Check sheet for the modelled part. Datum: model origin and axes. Units: mm. A direction names the side the tool comes from. Give positions to 0.01 mm unless a question says otherwise; leave off trailing zeros. Order: outer loops, then holes, each group sorted by start corner. A loop starts at its lowest first (then second) coordinate and runs counter-clockwise, first axis right, second up.
```python
from build123d import *

# Parameters (mm, degrees)
SKETCH2_R           = 5
BOSS_EXTRUDE1_DEPTH = 10.5
SKETCH3_R           = 2.5
CUT_EXTRUDE1_DEPTH  = 3.5
SKETCH4_R           = 1
CUT_EXTRUDE2_DEPTH  = 10.949874371
SKETCH5_W           = 1.25
SKETCH5_H           = 6
CUT_EXTRUDE3_DEPTH  = 16.33786165
SKETCH6_W           = 2.3
SKETCH6_H           = 6
CUT_EXTRUDE4_DEPTH  = 16.33786165
SKETCH7_R           = 2.6
CUT_EXTRUDE5_DEPTH  = 6
SKETCH8_R           = 0.5
CUT_EXTRUDE6_DEPTH  = 15.553779578


with BuildPart() as part:
    # Sketch2 → Boss-Extrude1 (new body)
    with BuildSketch(Plane.XY):
        with Locations(Location((0, 0, 0), (0, 0, 180))):
            Circle(SKETCH2_R)
    extrude(amount=BOSS_EXTRUDE1_DEPTH)

    # Sketch3 → Cut-Extrude1 (cut)
    with BuildSketch(Plane(origin=(0, 0, 0), x_dir=(-1, 0, 0), z_dir=(0, 0, -1))):
        Circle(SKETCH3_R)
    extrude(amount=-CUT_EXTRUDE1_DEPTH, mode=Mode.SUBTRACT)

    # Sketch4 → Cut-Extrude2 (cut, through all)
    with BuildSketch(Plane(origin=(0, 0, 3.5), x_dir=(-1, 0, 0), z_dir=(0, 0, -1))):
        Circle(SKETCH4_R)
    extrude(amount=-CUT_EXTRUDE2_DEPTH, mode=Mode.SUBTRACT)

    # Sketch5 → Cut-Extrude3 (cut, through all)
    with BuildSketch(Plane(origin=(0, 5, 0), x_dir=(1, 0, 0), z_dir=(0, 1, 0))):
        with Locations((-4.375, -7.5)):
            Rectangle(SKETCH5_W, SKETCH5_H)
        with Locations((4.375, -7.5)):
            Rectangle(SKETCH5_W, SKETCH5_H)
    extrude(amount=-CUT_EXTRUDE3_DEPTH, mode=Mode.SUBTRACT)

    # Sketch6 → Cut-Extrude4 (cut, through all)
    with BuildSketch(Plane(origin=(0, 5, 0), x_dir=(1, 0, 0), z_dir=(0, 1, 0))):
        with Locations((0, -7.5)):
            Rectangle(SKETCH6_W, SKETCH6_H)
    extrude(amount=-CUT_EXTRUDE4_DEPTH, mode=Mode.SUBTRACT)

    # Sketch7 → Cut-Extrude5 (cut)
    with BuildSketch(Plane.XY.offset(10.5)):
        Circle(SKETCH7_R)
    extrude(amount=-CUT_EXTRUDE5_DEPTH, mode=Mode.SUBTRACT)

    # Sketch8 → Cut-Extrude6 (cut, through all)
    with BuildSketch(Plane.ZY.offset(3.75)):
        with Locations((8, 1.85)):
            Circle(SKETCH8_R)
        with Locations((8, -1.85)):
            Circle(SKETCH8_R)
    extrude(amount=-CUT_EXTRUDE6_DEPTH, mode=Mode.SUBTRACT)


solid = part.part
```
Q1. Sectioned sample at B-B, the plane z = 9.5. Record the cut outline in (x, y), plus the area to 3 significant figures.
Q2. Material ranges on line 1 (Z direction, x = 2.6, y = -1.85); line 2 (Y direction, x = 0, z = 0.8); line 3 (X direction, y = -3, z = 8.5), recorded low to high.
Q3. Sectioned sample at C-C, the plane y = 0. Record the cut outline in (x, z), plus the area to 3 significant figures.
Q4. Sectioned sample at A-A, the plane x = 0. Record the cut outline in (y, z).
Q5. Tool access check on faces 4 (the flat face through (-3.75, 0, 8)), 5 (the cylindrical face through (-2.6, 0, 7.5)), 6 (the flat face through (1.15, 4, 8)), 7 (the flat face through (4, 0, 4.5)), 8 (the flat face through (-1, -1, 3.5)). Record the directions out of +Z, -Z, +X, -X, +Y, -Y that give a thin tool (end or side, any length) a straight path to the whole face; none if there is none.
Q6. Draft check along Y on faces 1 (the cylindrical face through (-3, -4, 4)), 2 (the flat face through (-3, 0, 10.5)), 3 (the cylindrical face through (2.721, 2.346, 7.935)). Enter one of: pulls with the +Y half, pulls with the -Y half, needs draft (parallel to the pull), parting line crosses it, or undercut.
Q7. Sectioned sample at D-D, the plane y = -1.85. Record the cut outline in (x, z).
Q8. Go/stop test with flat-tipped pins: P1, Ø1.4, axis at x = 4.5, y = 1.5, coming from the +Z side; P2, Ø2, axis at y = 4, z = 7.5, coming from the -X side; P3, Ø3, axis at y = 0, z = 7.5, coming from the +X side. Record where each tip stops, or that it passes through.
Filled in:
1. outline: (-3.75, -3.31) arc R5 ccw to (-1.15, -4.87) - (-1.15, -2.33) arc R2.6 cw to (-1.15, 2.33) - (-1.15, 4.87) arc R5 ccw to (-3.75, 3.31) - close; (1.15, -4.87) arc R5 ccw to (3.75, -3.31) - (3.75, 3.31) arc R5 ccw to (1.15, 4.87) - (1.15, 2.33) arc R2.6 cw to (1.15, -2.33) - close
1. area: 34.7 mm2
2. line 1: z = 0 to 7.5, 8.5 to 10.5
2. line 2: y = -5 to -2.5, 2.5 to 5
2. line 3: x = -3.75 to -1.15, 1.15 to 3.75
3. outline: (-5, 0) - (-2.5, 0) - (-2.5, 3.5) - (-1, 3.5) - (-1, 4.5) - (-2.6, 4.5) - (-2.6, 10.5) - (-3.75, 10.5) - (-3.75, 4.5) - (-5, 4.5) - close; (1, 3.5) - (2.5, 3.5) - (2.5, 0) - (5, 0) - (5, 4.5) - (3.75, 4.5) - (3.75, 10.5) - (2.6, 10.5) - (2.6, 4.5) - (1, 4.5) - close
3. area: 39.3 mm2
4. outline: (-5, 0) - (-2.5, 0) - (-2.5, 3.5) - (-1, 3.5) - (-1, 4.5) - (-5, 4.5) - close; (1, 3.5) - (2.5, 3.5) - (2.5, 0) - (5, 0) - (5, 4.5) - (1, 4.5) - close
5. face 4: +Z, -X, +Y, -Y
5. face 5: +Z
5. face 6: +Z, +Y, -Y
5. face 7: +Z, +X, +Y, -Y
5. face 8: -Z
6. face 1: parting line crosses it
6. face 2: needs draft
6. face 3: undercut
7. outline: (-4.65, 0) - (-1.68, 0) - (-1.68, 3.5) - (1.68, 3.5) - (1.68, 0) - (4.65, 0) - (4.65, 4.5) - (3.75, 4.5) - (3.75, 7.5) - (1.83, 7.5) - (1.83, 4.5) - (-1.83, 4.5) - (-1.83, 7.5) - (-3.75, 7.5) - (-3.75, 4.5) - (-4.65, 4.5) - close; (-3.75, 8.5) - (-1.83, 8.5) - (-1.83, 10.5) - (-3.75, 10.5) - close; (1.83, 8.5) - (3.75, 8.5) - (3.75, 10.5) - (1.83, 10.5) - close
8. P1: stops at z = 4.5
8. P2: stops at x = -3.75
8. P3: stops at x = 3.75
